Verification items for the finished model (mm, model axes). Coordinates: 2 decimals unless noted, no trailing zeros. Write each loop counter-clockwise with the first axis right and the second up, starting at its lowest first coordinate (ties: lowest second). Pieces come first, ordered by that corner, then holes. Notation, with made-up numbers: (26.25, -27) -> (68.25, -27) arc R32 cw to (68.25, 11) -> close; hole circle Ø8 at (80.25, 40). An arc over 180 degrees is marked (long way). Use CSV: the item, a comma, the result in double quotes.
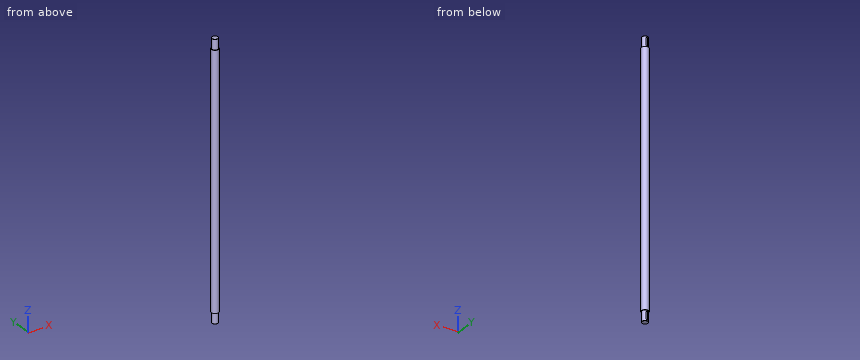
```python
from build123d import *

# Parameters (mm, degrees)
SKETCH1_R                = 30
EXTRUDE1_DEPTH           = 1033.5
SKETCH2_R                = 25
EXTRUDE2_DEPTH           = 84
CHAMFER1_SIZE            = 1
EXTRUDE3_DEPTH           = 5.5
CHAMFER1_OF_MIRROR1_SIZE = 1


with BuildPart() as part:
    # Sketch1 → Extrude1 (new, symmetric)
    with BuildSketch(Plane.XY):
        Circle(SKETCH1_R)
    extrude(amount=EXTRUDE1_DEPTH, both=True)

    # Sketch2 → Extrude2 (add)
    with BuildSketch(Plane.XY.offset(1033.5)):
        with Locations(Location((0, 0, 0), (0, 0, 180))):
            Circle(SKETCH2_R)
    extrude2 = extrude(amount=EXTRUDE2_DEPTH)

    # Chamfer1
    chamfer1_edges = [part.edges().sort_by_distance(p)[0] for p in [
        (25, 0, 1117.5),
    ]]
    chamfer(chamfer1_edges, length=CHAMFER1_SIZE)

    # Sketch3 → Extrude3 (cut)
    with BuildSketch(Plane(origin=(0, 19.5, 0), x_dir=(-1, 0, 0), z_dir=(0, 1, 0))):
        with BuildLine():
            Line((7, 1102.5), (7, 1046.5))
            ThreePointArc((7, 1046.5), (0, 1039.5), (-7, 1046.5))
            Line((-7, 1046.5), (-7, 1102.5))
            ThreePointArc((-7, 1102.5), (0, 1109.5), (7, 1102.5))
        make_face()
    extrude3 = extrude(amount=EXTRUDE3_DEPTH, mode=Mode.SUBTRACT)

    # Mirror1: Extrude2, Extrude3 across plane
    add(extrude2.mirror(Plane.XY))
    add(extrude3.mirror(Plane.XY), mode=Mode.SUBTRACT)

    # Chamfer1 of Mirror1
    chamfer1_of_mirror1_edges = [part.edges().sort_by_distance(p)[0] for p in [
        (25, 0, -1117.5),
    ]]
    chamfer(chamfer1_of_mirror1_edges, length=CHAMFER1_OF_MIRROR1_SIZE)


solid = part.part
```
1) Gauge pin test, flat ends, axial feed: pin 1 (2 mm diameter, centred on y = 22.5, z = -1075, fed in from -X); pin 2 (4 mm diameter, centred on x = 12, z = -140.5, fed in from -Y); pin 3 (15.5 mm diameter, centred on x = 1.5, z = 1067.5, fed in from +Y). Record the tip position at first contact, or that the pin passes through.
Return value:
pin 1,"x = -12.76"
pin 2,"y = -28.28"
pin 3,"y = 24"
2) Cross-section at A-A (z = -38.5). Record the boundary of the cut face in (x, y), plus the area to 3 significant figures.
Return value:
outline,"circle Ø60 at (0, 0)"
area,"2,830 mm2"
3) Scan lines: L1, parallel to Z at x = 10, y = -27; L2, parallel to Y at x = -17, z = 797.5; L3, parallel to X at y = 2.5, z = -493.5. Record each from-to range of solid material in increasing order.
Return value:
L1,"-1033.5 to 1033.5"
L2,"-24.72 to 24.72"
L3,"-29.9 to 29.9"
